from build123d import *

# Parameters (mm, degrees)
SKETCH_1_W          = 120
SKETCH_1_H          = 88
SKETCH_1_R          = 1.65
SKETCH_1_R_2        = 2.5
EXTRUDE_1_DEPTH     = 1
SKETCH_2_R          = 4.5
CUT_EXTRUDE_1_DEPTH = 2.5


with BuildPart() as part:
    # 草图1 → 凸台-拉伸1 (new, symmetric)
    with BuildSketch(Plane.XY):
        Rectangle(SKETCH_1_W, SKETCH_1_H)
        with Locations((-40, -22.5)):
            Circle(SKETCH_1_R, mode=Mode.SUBTRACT)
        with Locations((-40, 22.5)):
            Circle(SKETCH_1_R, mode=Mode.SUBTRACT)
        with Locations((40, -22.5)):
            Circle(SKETCH_1_R, mode=Mode.SUBTRACT)
        with Locations((40, 22.5)):
            Circle(SKETCH_1_R, mode=Mode.SUBTRACT)
        with Locations((-50, -35)):
            Circle(SKETCH_1_R, mode=Mode.SUBTRACT)
        with Locations((-50, 35)):
            Circle(SKETCH_1_R, mode=Mode.SUBTRACT)
        with Locations((50, -35)):
            Circle(SKETCH_1_R, mode=Mode.SUBTRACT)
        with Locations((50, 35)):
            Circle(SKETCH_1_R, mode=Mode.SUBTRACT)
        with Locations((-24, 35)):
            Circle(SKETCH_1_R_2, mode=Mode.SUBTRACT)
    extrude(amount=EXTRUDE_1_DEPTH, both=True)

    # 草图2 → 切除-拉伸1 (cut, symmetric)
    with BuildSketch(Plane.XY):
        with Locations((-62, -47)):
            Circle(SKETCH_2_R)
        with Locations((-62, 47)):
            Circle(SKETCH_2_R)
        with Locations((62, -47)):
            Circle(SKETCH_2_R)
        with Locations((62, 47)):
            Circle(SKETCH_2_R)
    extrude(amount=CUT_EXTRUDE_1_DEPTH, both=True, mode=Mode.SUBTRACT)


solid = part.part
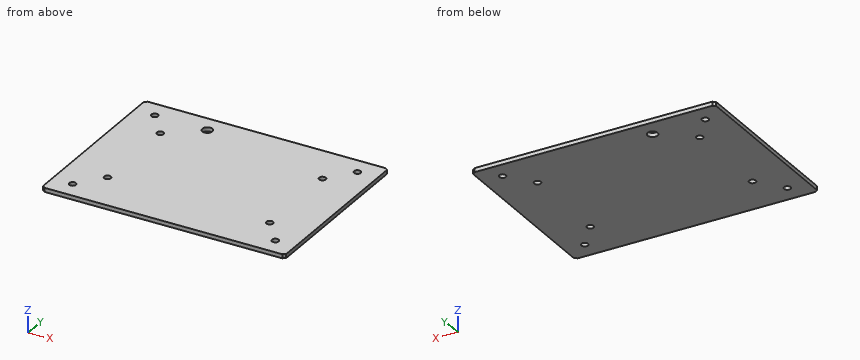
The listing builds one solid part. Answer for the finished solid, in the listing's coordinates (mm). Coordinates: 2 decimals unless noted, no trailing zeros. Loops run counter-clockwise (first coordinate to the right, second up) from the corner with the lowest first, then second, coordinate; pieces in that order, holes last. Notation, with made-up numbers: (-34.5, -12) -> (0.5, -12) arc R34 ccw to (0.5, 27) -> close; hole circle Ø1 at (53.5, -24). An arc over 180 degrees is marked (long way). Write item = value, one per line. Start each with the question number.
1) A cutting plane is placed at A-A (y = 35). Give the vertices of the cut face in (x, z), then the cut area to 3 significant figures.
2) A cutting plane is placed at B-B (x = -50). Give the vertices of the cut face in (y, z), then the cut area to 3 significant figures.
3) Straight lines are drawn through the part: line 1 (Y direction, x = -50, z = 0.35); line 2 (Y direction, x = 40, z = 0.2). For each, find the intervals that lie inside material, in ascending order. Write a range as from..to.
4) A cutting plane is placed at C-C (y = -35). Give the vertices of the cut face in (x, z).
Responses:
q1.outline = (-60, -1) -> (-51.65, -1) -> (-51.65, 1) -> (-60, 1) -> close; (-48.35, -1) -> (-26.5, -1) -> (-26.5, 1) -> (-48.35, 1) -> close; (-21.5, -1) -> (48.35, -1) -> (48.35, 1) -> (-21.5, 1) -> close; (51.65, -1) -> (60, -1) -> (60, 1) -> (51.65, 1) -> close
q1.area = 217 mm²
q2.outline = (-44, -1) -> (-36.65, -1) -> (-36.65, 1) -> (-44, 1) -> close; (-33.35, -1) -> (33.35, -1) -> (33.35, 1) -> (-33.35, 1) -> close; (36.65, -1) -> (44, -1) -> (44, 1) -> (36.65, 1) -> close
q2.area = 163 mm²
q3.line_1 = -44..-36.65, -33.35..33.35, 36.65..44
q3.line_2 = -44..-24.15, -20.85..20.85, 24.15..44
q4.outline = (-60, -1) -> (-51.65, -1) -> (-51.65, 1) -> (-60, 1) -> close; (-48.35, -1) -> (48.35, -1) -> (48.35, 1) -> (-48.35, 1) -> close; (51.65, -1) -> (60, -1) -> (60, 1) -> (51.65, 1) -> close
